For this review, take the finished solid that the model builds, in its own axes (mm). A direction names the side the tool comes from. Coordinates: 2 decimals unless noted, no trailing zeros. Loops run counter-clockwise (first coordinate to the right, second up) from the corner with the lowest first, then second, coordinate; pieces in that order, holes last.
1. Machinability: for faces 1 (the face through (-0.225, -3.451, 0.715)), 2 (the face through (0.338, 36.827, 1.073)), 3 (the face through (0.225, 78.249, 0.715)), which of the approach directions +Z, -Z, +X, -X, +Y, -Y give a long, thin tool a straight path to every point of the face, cutting with its end or side? Answer none if there is none.
2. To check wall thickness, follow probe 1 along Y at (x, z) = (0.1, 1.05); probe 2 along Y at (x, z) = (-0.2, -0.55); probe 3 along Z at (x, y) = (-0.2, 56.5). State the ranges of each line that lie inside material, in increasing order.
3. Take a section at A-A, the plane y = 59. State the section outline as (x, z) points (3 decimals).
```python
from build123d import *

# Parameters (mm, degrees)
SKETCH1_R           = 1.125
BOSS_EXTRUDE1_DEPTH = 74.7
SKETCH2_R           = 0.75
BOSS_EXTRUDE2_DEPTH = 7
SKETCH3_R           = 0.3
BOSS_EXTRUDE3_DEPTH = 3.5
BOSS_EXTRUDE4_START = 7
SKETCH4_R           = 0.75
BOSS_EXTRUDE4_DEPTH = 7
SKETCH5_R           = 0.299867591
BOSS_EXTRUDE5_DEPTH = 3


with BuildPart() as part:
    # Sketch1 → Boss-Extrude1 (new body)
    with BuildSketch(Plane(origin=(0, 0, 0), x_dir=(1, 0, 0), z_dir=(0, 1, 0))):
        with Locations(Location((0, 0, 0), (0, 0, 270))):
            Circle(SKETCH1_R)
    extrude(amount=BOSS_EXTRUDE1_DEPTH)

    # Sketch2 → Boss-Extrude2 (add)
    with BuildSketch(Plane.XZ):
        with Locations(Location((0, 0, 0), (0, 0, 90))):
            Circle(SKETCH2_R)
    extrude(amount=BOSS_EXTRUDE2_DEPTH)

    # Sketch3 → Boss-Extrude3 (add)
    with BuildSketch(Plane.XZ.offset(7)):
        with Locations(Location((0, 0, 0), (0, 0, 270))):
            Circle(SKETCH3_R)
    extrude(amount=BOSS_EXTRUDE3_DEPTH)

    # Sketch4 → Boss-Extrude4 (add)
    with BuildSketch(Plane(origin=(0, 74.7, 0), x_dir=(1, 0, 0), z_dir=(0, 1, 0)).offset(BOSS_EXTRUDE4_START)):
        with Locations(Location((0, 0, 0), (0, 0, 270))):
            Circle(SKETCH4_R)
    extrude(amount=-BOSS_EXTRUDE4_DEPTH)

    # Sketch5 → Boss-Extrude5 (add)
    with BuildSketch(Plane(origin=(0, 81.7, 0), x_dir=(1, 0, 0), z_dir=(0, 1, 0))):
        with Locations(Location((0, 0, 0), (0, 0, 270))):
            Circle(SKETCH5_R)
    extrude(amount=BOSS_EXTRUDE5_DEPTH)


solid = part.part
```
Results list:
1. face 1: -Y
1. face 2: +Y, -Y
1. face 3: +Y
2. probe 1: y = 0 to 74.7
2. probe 2: y = -7 to 81.7
2. probe 3: z = -1.11 to 1.11
3. outline: circle Ø2.25 at (0, 0)
